The listing builds one solid part. Answer for the finished solid, in the listing's coordinates (mm). A direction names the side the tool comes from. Coordinates: 2 decimals unless noted, no trailing zeros. Order: outer loops, then holes, each group sorted by start corner. A loop starts at its lowest first (then second) coordinate and runs counter-clockwise, first axis right, second up. Notation, with made-up numbers: (-28, 40) -> (28, 40) arc R9 cw to (28, 46) -> close; hole circle Ø4 at (71.5, 81.5). An arc over 180 degrees is marked (long way). Write item = value, one per line.
from build123d import *

# Parameters (mm, degrees)
SKETCH_1_W             = 150
SKETCH_1_H             = 150
EXTRUDE_1_DEPTH        = 5
SKETCH_3_R             = 17.5
CUT_EXTRUDE_1_DEPTH    = 107.536378763
HOLE_WIZARD_M5_1_D     = 5.8
CHAMFER_1_SIZE         = 2
SKETCH_6_R             = 35
CUT_EXTRUDE_2_DEPTH    = 5
HOLE_WIZARD_M6_1_D     = 5
HOLE_WIZARD_M6_1_DEPTH = 10
HOLE_WIZARD_M5_1_2_D   = 4.2


with BuildPart() as part:
    # 草图1 → 凸台-拉伸1 (new, symmetric)
    with BuildSketch(Plane.XY):
        Rectangle(SKETCH_1_W, SKETCH_1_H)
    extrude(amount=EXTRUDE_1_DEPTH, both=True)

    # 草图3 → 切除-拉伸1 (cut, through all)
    with BuildSketch(Plane(origin=(0, 0, -5), x_dir=(-1, 0, 0), z_dir=(0, 0, -1))):
        with Locations((0, -1)):
            Circle(SKETCH_3_R)
    extrude(amount=-CUT_EXTRUDE_1_DEPTH, mode=Mode.SUBTRACT)

    # Hole Wizard M5 _1 (through all)
    with Locations(Plane(origin=(0, 0, -5), x_dir=(-1, 0, 0), z_dir=(0, 0, -1))):
        with Locations((-70, 70), (-70, 0), (-70, -70), (0, -70), (70, -70), (70, 0), (70, 70), (0, 70)):
            Hole(HOLE_WIZARD_M5_1_D / 2)

    # 倒角1
    chamfer_1_edges = [part.edges().sort_by_distance(p)[0] for p in [
        (75, -75, 0),
        (-75, -75, 0),
        (-75, 75, 0),
        (75, 75, 0),
    ]]
    chamfer(chamfer_1_edges, length=CHAMFER_1_SIZE)

    # 草图6 → 切除-拉伸2 (cut)
    with BuildSketch(Plane.XY.offset(5)):
        with Locations((0, -1)):
            Circle(SKETCH_6_R)
    extrude(amount=-CUT_EXTRUDE_2_DEPTH, mode=Mode.SUBTRACT)

    # M6 螺纹孔1
    with Locations(Plane.XY.offset(5)):
        with Locations((-36.06, 35.06), (0, -1), (36.06, -37.06), (36.06, 35.06), (-36.06, -37.06)):
            Hole(HOLE_WIZARD_M6_1_D / 2, depth=HOLE_WIZARD_M6_1_DEPTH)

    # Hole Wizard M5 _1 2 (through all)
    with Locations(Plane(origin=(0, 0, -5), x_dir=(-1, 0, 0), z_dir=(0, 0, -1))):
        with Locations((-30, 26), (30, 26), (-30, -28), (30, -28)):
            Hole(HOLE_WIZARD_M5_1_2_D / 2)


solid = part.part
Q1. Section C-C, the plane y = -7.5 is taken. Give the vertices of the cut face in (x, z), plus the area to 3 significant figures.
The answers:
outline = (-75, -5) -> (-16.25, -5) -> (-16.25, 0) -> (-34.39, 0) -> (-34.39, 5) -> (-75, 5) -> close; (16.25, -5) -> (75, -5) -> (75, 5) -> (34.39, 5) -> (34.39, 0) -> (16.25, 0) -> close
area = 994 mm2
Q2. Section A-A, the plane y = -70 is taken. Give the vertices of the cut face in (x, z), plus the area to 3 significant figures.
The answers:
outline = (-75, -5) -> (-72.9, -5) -> (-72.9, 5) -> (-75, 5) -> close; (-67.1, -5) -> (-2.9, -5) -> (-2.9, 5) -> (-67.1, 5) -> close; (2.9, -5) -> (67.1, -5) -> (67.1, 5) -> (2.9, 5) -> close; (72.9, -5) -> (75, -5) -> (75, 5) -> (72.9, 5) -> close
area = 1,330 mm2
Q3. Section D-D, the plane x = -23 is taken. Give the vertices of the cut face in (y, z), plus the area to 3 significant figures.
The answers:
outline = (-75, -5) -> (75, -5) -> (75, 5) -> (25.38, 5) -> (25.38, 0) -> (-27.38, 0) -> (-27.38, 5) -> (-75, 5) -> close
area = 1,240 mm2
Q4. Section B-B, the plane z = -2.5 is taken. Give the number of separate pieces and of enclosed holes in the cut face, plus the area to 3 significant figures.
The answers:
separate_pieces = 1
enclosed_holes = 17
area = 21,200 mm2
Q5. The mould has two halves that part along Y. Classify faces 1 (the face through (67.1, 0.1, 0.1)), 2 (the face through (-1, -75, 0)), 3 (the face through (-1, 18, -5)), 4 (the face through (67.699, -71.765, 0.07)): released by +Y, released by -Y, zero draft, split by the parting line, or undercut.
The answers:
face_1 = undercut
face_2 = released by -Y
face_3 = zero draft
face_4 = undercut
Q6. Each of these flat-tipped pins is pushed along its axis until it touches: pin 1 Ø4.5 at (x, y) = (-70, 0) entering from +Z; pin 2 Ø6 at (x, y) = (14, 8) entering from +Z. Where does it stop, or does it pass through?
The answers:
pin_1 = through
pin_2 = 0
Q7. A tool of negligible diameter and unlimited length cuts with its end or side. For faces 5 (the face through (27.9, -27.91, 0.07)), 6 (the face through (-8, 15, 0)), from which of +Z, -Z, +X, -X, +Y, -Y can it reach the whole face along a straight path? Write none if from no direction.
The answers:
face_5 = +Z, -Z
face_6 = +Z
Q8. Find the intervals of material crossed by line 1 along Y through (x, z) = (70, -0.75); line 2 along Y through (x, z) = (0, 2.75); line 3 along Y through (x, z) = (36.06, -0.5), in increasing order.
The answers:
line_1 = -75 to -72.9, -67.1 to -2.9, 2.9 to 67.1, 72.9 to 75
line_2 = -75 to -72.9, -67.1 to -36, 34 to 67.1, 72.9 to 75
line_3 = -75 to -39.56, -34.56 to 32.56, 37.56 to 75
